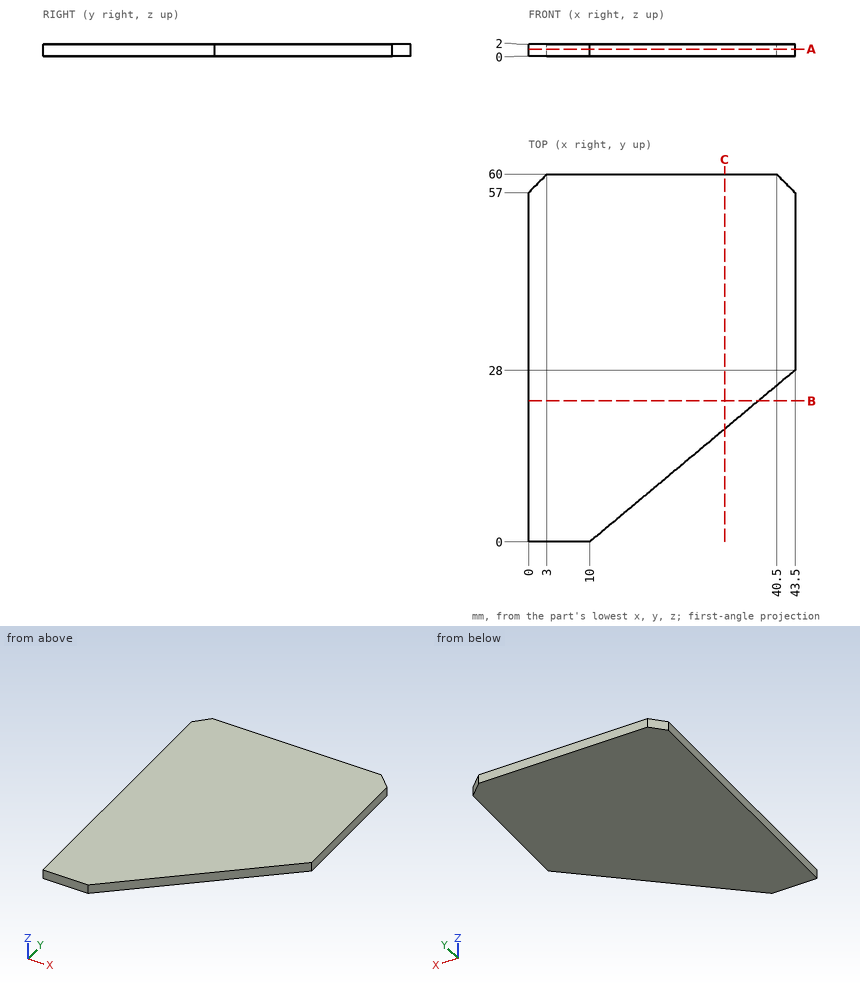
Part print with two shaded views. Sizes in mm from the minimum x, y, z corner. Round coordinates to 2 decimals unless told otherwise and drop trailing zeros. Write each loop counter-clockwise with the first axis right and the second up, starting at its lowest first coordinate (ties: lowest second). Pieces come first, ordered by that corner, then holes. Notation, with made-up numbers: (64.25, 87.5) - (89.25, 87.5) arc R25 ccw to (89.25, 107.5) - close; hole circle Ø2 at (-23.5, -8.5). An arc over 180 degrees is marked (long way). Use CSV: the item, a comma, the result in double quotes.
Item 1: Slice it at B-B, the plane y = 23. Write the cut outline in (x, z), then the cut area to 3 significant figures.
Results list:
outline,"(0, 0) - (37.52, 0) - (37.52, 2) - (0, 2) - close"
area,"75.0 mm²"
Item 2: Slice it at A-A, the plane z = 1.15. Write the cut outline in (x, y).
Results list:
outline,"(0, 0) - (10, 0) - (43.5, 28) - (43.5, 57) - (40.5, 60) - (3, 60) - (0, 57) - close"
Item 3: Wall check: L1, parallel to Y at x = 37, z = 0.15; L2, parallel to X at y = 19, z = 1.05; L3, parallel to Y at x = 37.5, z = 0.25. Give the ranges that are in metal, low to high.
Results list:
L1,"y = 22.57 to 60"
L2,"x = 0 to 32.73"
L3,"y = 22.99 to 60"
Item 4: Slice it at C-C, the plane x = 32. Write the cut outline in (y, z).
Results list:
outline,"(18.39, 0) - (60, 0) - (60, 2) - (18.39, 2) - close"
